Model file for the job. Use its own axes, mm. Face numbers are marked on the shaded views. A direction names the side the tool comes from. Round coordinates to 2 decimals unless told otherwise and drop trailing zeros. Order: outer loops, then holes, each group sorted by start corner. A loop starts at its lowest first (then second) coordinate and runs counter-clockwise, first axis right, second up. Notation, with made-up numbers: (48, -29) - (62, -29) arc R36 ccw to (62, 7) - close; hole circle Ø2 at (38.5, -27.5). An arc over 180 degrees is marked (long way). Answer as CSV lines item,"result". Start each with the question number.
1. Band-saw the part on B-B on y = 78.5. List the corners of the cut face in (x, z), then the cut area to 3 significant figures.
2. Band-saw the part on A-A on x = 104. List the corners of the cut face in (y, z).
3. Pull direction Y, two halves, no side cores. Call the marked faces 1, 2 and 3: released by +Y, released by -Y, zero draft, split by the parting line, or undercut.
4. Band-saw the part on C-C on z = 14.5. State how many separate pieces and enclosed holes the cut face has, then the cut area to 3 significant figures.
5. 3-axis set-ups, long thin cutter, end or side, ignore diameter. For the marked faces 4, 5 and 6: which of +Z, -Z, +X, -X, +Y, -Y reach the whole face in a straight line?
6. Pin check, flat tips, straight feed: pin 1 Ø4.5 at (x, z) = (83, 7) entering from -Y; pin 2 Ø6 at (y, z) = (75.5, 8.5) entering from -X; pin 3 Ø21 at (x, z) = (65, 20) entering from +Y; pin 4 Ø3 at (x, z) = (45, 20) entering from -Y. Stop position of each tip, or through.
7. Wall check: line 1 along Y through (x, z) = (140, 17); line 2 along X through (y, z) = (9.5, 33); line 3 along Y through (x, z) = (141, 29.5). Give the ranges that are in metal, low to high. Write a range as [from, to].
```python
from build123d import *

# Parameters (mm, degrees)
BOSS_EXTRUDE1_DEPTH   = 40
SKETCH2_R             = 11
CUT_EXTRUDE1_DEPTH    = 190.1137224
SKETCH3_R             = 13
CUT_EXTRUDE2_DEPTH    = 40
SKETCH4_R             = 11.85
CUT_EXTRUDE3_DEPTH    = 1.1
SKETCH5_R             = 13.5
CUT_EXTRUDE4_DEPTH    = 1.3
LPATTERN1_COUNT       = 2
LPATTERN1_PITCH       = 7.3
M3_TAPPED_HOLE1_D     = 2.5
M3_TAPPED_HOLE1_DEPTH = 7.5
M3_TAPPED_HOLE1_TIP   = 0.751075774
CUT_EXTRUDE5_REACH    = 191.114
CHAMFER1_SIZE         = 0.5
M3_TAPPED_HOLE2_D     = 2.5
M3_TAPPED_HOLE2_DEPTH = 7.5
M3_TAPPED_HOLE2_TIP   = 0.751075774
M4_TAPPED_HOLE1_D     = 3.3
M4_TAPPED_HOLE1_DEPTH = 15.5
M4_TAPPED_HOLE1_TIP   = 0.991420021
SKETCH14_R            = 2.25
CUT_EXTRUDE6_DEPTH    = 24
M4_TAPPED_HOLE2_D     = 3.3
M4_TAPPED_HOLE2_DEPTH = 15


with BuildPart() as part:
    # Sketch1 → Boss-Extrude1 (new body)
    with BuildSketch(Plane.XY):
        with BuildLine():
            Line((0, 0), (141, 0))
            ThreePointArc((141, 0), (147.363961031, 2.636038969), (150, 9))
            Line((150, 9), (150, 99))
            ThreePointArc((150, 99), (147.363961031, 105.363961031), (141, 108))
            Line((141, 108), (0, 108))
            Line((0, 108), (0, 93))
            Line((0, 93), (121, 93))
            ThreePointArc((121, 93), (127.363961031, 90.363961031), (130, 84))
            Line((130, 84), (130, 24))
            ThreePointArc((130, 24), (127.363961031, 17.636038969), (121, 15))
            Line((121, 15), (0, 15))
            Line((0, 15), (0, 0))
        make_face()
    extrude(amount=BOSS_EXTRUDE1_DEPTH)

    # Sketch2 → Cut-Extrude1 (cut, through all)
    with BuildSketch(Plane(origin=(0, 108, 0), x_dir=(1, 0, 0), z_dir=(0, 1, 0))):
        with Locations(Location((65, -20, 0), (0, 0, 180))):
            Circle(SKETCH2_R)
    extrude(amount=-CUT_EXTRUDE1_DEPTH, mode=Mode.SUBTRACT)

    # Sketch3 → Cut-Extrude2 (cut)
    with BuildSketch(Plane(origin=(0, 108, 0), x_dir=(1, 0, 0), z_dir=(0, 1, 0))):
        with Locations(Location((65, -20, 0), (0, 0, 180))):
            Circle(SKETCH3_R)
    extrude(amount=-CUT_EXTRUDE2_DEPTH, mode=Mode.SUBTRACT)

    # Sketch4 → Cut-Extrude3 (cut)
    with BuildSketch(Plane(origin=(0, 12, 0), x_dir=(1, 0, 0), z_dir=(0, 1, 0))):
        with Locations(Location((65, -20, 0), (0, 0, 180))):
            Circle(SKETCH4_R)
    extrude(amount=CUT_EXTRUDE3_DEPTH, mode=Mode.SUBTRACT)

    # Sketch5 → Cut-Extrude4 (cut)
    with BuildSketch(Plane(origin=(0, 96, 0), x_dir=(-1, 0, 0), z_dir=(0, -1, 0))):
        with Locations(Location((-65, -20, 0), (0, 0, 90))):
            Circle(SKETCH5_R)
    cut_extrude4 = extrude(amount=CUT_EXTRUDE4_DEPTH, mode=Mode.SUBTRACT)

    # LPattern1: Cut-Extrude4 ×2
    with Locations(*[(0, i * LPATTERN1_PITCH, 0) for i in range(1, LPATTERN1_COUNT)]):
        add(cut_extrude4, mode=Mode.SUBTRACT)

    # M3 Tapped Hole1
    with Locations(Plane(origin=(45, 108, 20), x_dir=(1, 0, 0), z_dir=(0, 1, 0))):
        with Locations((0, 0), (40, 0)):
            Hole(M3_TAPPED_HOLE1_D / 2, depth=M3_TAPPED_HOLE1_DEPTH)
            with Locations((0, 0, -(M3_TAPPED_HOLE1_DEPTH + M3_TAPPED_HOLE1_TIP / 2))):  # 118° drill point
                Cone(0, M3_TAPPED_HOLE1_D / 2, M3_TAPPED_HOLE1_TIP, mode=Mode.SUBTRACT)

    # Sketch9 → Cut-Extrude5 (cut, up to next)
    with BuildSketch(Plane(origin=(150, 0, 0), x_dir=(0, 0, -1), z_dir=(1, 0, 0)), mode=Mode.PRIVATE) as cut_extrude5_sk1:
        Polygon((-40, 24), (-30, 34), (-20, 34), (-20, 74), (-30, 74), (-40, 84), align=None)
    cut_extrude5_tool1 = extrude(cut_extrude5_sk1.sketch, amount=-CUT_EXTRUDE5_REACH, mode=Mode.PRIVATE) & part.part
    add(cut_extrude5_tool1.solids().sort_by_distance((150, 54, 30.740741))[0], mode=Mode.SUBTRACT)

    # Chamfer1
    chamfer1_edges = [part.edges().sort_by_distance(p)[0] for p in [
        (76, 0, 20),
        (76, 15, 20),
        (78, 93, 20),
        (78, 108, 20),
    ]]
    chamfer(chamfer1_edges, length=CHAMFER1_SIZE)

    # M3 Tapped Hole2
    with Locations(Plane(origin=(140, 69, 20), x_dir=(1, 0, 0), z_dir=(0, 0, 1))):
        with Locations((0, 0), (0, -30)):
            Hole(M3_TAPPED_HOLE2_D / 2, depth=M3_TAPPED_HOLE2_DEPTH)
            with Locations((0, 0, -(M3_TAPPED_HOLE2_DEPTH + M3_TAPPED_HOLE2_TIP / 2))):  # 118° drill point
                Cone(0, M3_TAPPED_HOLE2_D / 2, M3_TAPPED_HOLE2_TIP, mode=Mode.SUBTRACT)

    # M4 Tapped Hole1
    with Locations(Plane(origin=(150, 17.860571099, 20), x_dir=(0, 0, 1), z_dir=(1, 0, 0))):
        with Locations((0, 0)):
            Hole(M4_TAPPED_HOLE1_D / 2, depth=M4_TAPPED_HOLE1_DEPTH)
            with Locations((0, 0, -(M4_TAPPED_HOLE1_DEPTH + M4_TAPPED_HOLE1_TIP / 2))):  # 118° drill point
                Cone(0, M4_TAPPED_HOLE1_D / 2, M4_TAPPED_HOLE1_TIP, mode=Mode.SUBTRACT)

    # Sketch14 → Cut-Extrude6 (cut)
    with BuildSketch(Plane.XZ):
        with Locations((85, 20)):
            Circle(SKETCH14_R)
        with Locations(Location((45, 20, 0), (0, 0, 270))):
            Circle(SKETCH14_R)
    extrude(amount=-CUT_EXTRUDE6_DEPTH, mode=Mode.SUBTRACT)

    # M4 Tapped Hole2
    with Locations(Plane(origin=(47, 0, 33), x_dir=(0, 0, -1), z_dir=(0, -1, 0))):
        with Locations((0, 0), (0, 36), (26, 36), (26, 0)):
            Hole(M4_TAPPED_HOLE2_D / 2, depth=M4_TAPPED_HOLE2_DEPTH)


solid = part.part
```
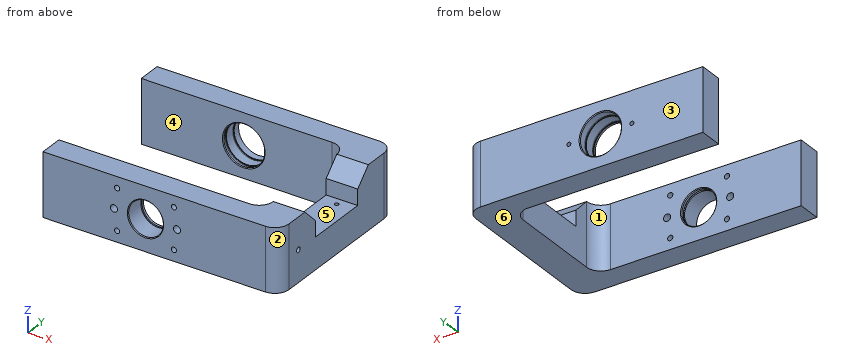
Reply:
1,outline,"(130, 0) - (150, 0) - (150, 34.5) - (130, 34.5) - close"
1,area,"690 mm2"
2,outline,"(0, 0) - (15, 0) - (15, 40) - (0, 40) - close; (93, 0) - (108, 0) - (108, 40) - (93, 40) - close"
3,face 1,"undercut"
3,face 2,"released by -Y"
3,face 3,"released by +Y"
4,separate pieces,"3"
4,enclosed holes,"2"
4,area,"5,400 mm2"
5,face 4,"+Z, -Z, -X"
5,face 5,"+Z, +X, -X"
5,face 6,"-Z, +X, -X, +Y, -Y"
6,pin 1,"stops at y = 0"
6,pin 2,"stops at x = 130"
6,pin 3,"passes through"
6,pin 4,"stops at y = 93"
7,line 1,"y = [0, 37.75], [40.25, 67.75], [70.25, 108]"
7,line 2,"x = [0, 45.35], [48.65, 81.35], [84.65, 150]"
7,line 3,"y = [0, 34], [74, 108]"
